CAD build for the part. Positions are in the model's coordinates, mm. Face numbers are marked on the shaded views. A direction names the side the tool comes from. Give positions to 0.01 mm unless a question says otherwise; leave off trailing zeros. Loops run counter-clockwise (first coordinate to the right, second up) from the corner with the lowest first, then second, coordinate; pieces in that order, holes last. Notation, with made-up numbers: (-39.5, 16.25) -> (-27.5, 16.25) arc R28 cw to (-27.5, 42.25) -> close; hole circle Ø3 at (15, 35). An arc over 180 degrees is marked (long way). Write each question's results on one line, items separated by ' | '. Start each with the question number.
```python
from build123d import *

# Parameters (mm, degrees)
HEAD_PROFILE_24X24_W      = 24
HEAD_PROFILE_24X24_H      = 24
SQUARE_HEAD_24X24X8_DEPTH = 8
SHANK_PROFILE_12_R        = 6
SHANK_12X104_DEPTH        = 104


with BuildPart() as part:
    # Head Profile 24x24 → Square Head 24x24x8 (new body)
    with BuildSketch(Plane(origin=(0, 0, 0), x_dir=(1, 0, 0), z_dir=(0, 1, 0))):
        Rectangle(HEAD_PROFILE_24X24_W, HEAD_PROFILE_24X24_H)
    extrude(amount=SQUARE_HEAD_24X24X8_DEPTH)

    # Shank Profile Ø12 → Shank Ø12x104 (add)
    with BuildSketch(Plane.XZ):
        with Locations(Location((0, 0, 0), (0, 0, 90))):
            Circle(SHANK_PROFILE_12_R)
    extrude(amount=SHANK_12X104_DEPTH)


solid = part.part
```
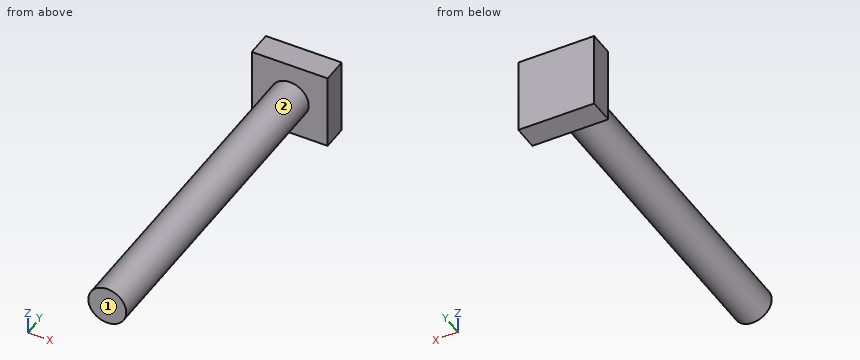
Q1. Drop flat-ended pins along their axis: pin 1 (1 mm diameter, centred on y = -73.5, z = -3, fed in from +X); pin 2 (6 mm diameter, centred on x = 2, y = -38, fed in from -Z); pin 3 (3 mm diameter, centred on y = -70.5, z = 6, fed in from +X). Give the stop position or say it passes through.
Q2. Which spindle directions (+Z, -Z, +X, -X, +Y, -Y) get a long thin tool onto all of the face, cutting with end or side? Do the marked faces 1 and 2. Say none if no direction does.
Q3. Wall check: L1, parallel to Y at x = -2.5, z = -6.5; L2, parallel to X at y = -7, z = 2.5; L3, parallel to X at y = -94, z = 3.25. Give the ranges that are in metal, low to high.
Q4. Saw through at A-A, the plane x = 0. List the corners of the cut face in (y, z), then the cut area to 3 significant figures.
Q5. Saw through at B-B, the plane z = 0. List the corners of the cut face in (x, y), then the cut area to 3 significant figures.
Q6. Saw through at C-C, the plane y = -49. List the corners of the cut face in (x, z), then the cut area to 3 significant figures.
Q7. Saw through at D-D, the plane x = 7.5. List the corners of the cut face in (y, z), then the cut area to 3 significant figures.
Answer block:
1) pin 1: stops at x = 5.45 | pin 2: stops at z = -6 | pin 3: stops at x = 3.97
2) face 1: +Z, -Z, +X, -X, -Y | face 2: -Y
3) L1: y = 0 to 8 | L2: x = -5.45 to 5.45 | L3: x = -5.04 to 5.04
4) outline: (-104, -6) -> (0, -6) -> (0, -12) -> (8, -12) -> (8, 12) -> (0, 12) -> (0, 6) -> (-104, 6) -> close | area: 1,440 mm2
5) outline: (-12, 0) -> (-6, 0) -> (-6, -104) -> (6, -104) -> (6, 0) -> (12, 0) -> (12, 8) -> (-12, 8) -> close | area: 1,440 mm2
6) outline: circle Ø12 at (0, 0) | area: 113 mm2
7) outline: (0, -12) -> (8, -12) -> (8, 12) -> (0, 12) -> close | area: 192 mm2
